Input: part model. Units: mm. Frame: model coordinates. Face numbers are marked on the shaded views. A direction names the side the tool comes from. Coordinates: 2 decimals unless noted, no trailing zeros. Write each loop counter-clockwise with the first axis right and the second up, starting at its lowest first coordinate (ties: lowest second). Pieces come first, ordered by that corner, then holes. Notation, with made-up numbers: (66, 42) - (100, 42) arc R23 cw to (100, 51) - close; hole circle Ø10 at (-5.5, -25.5). An arc over 180 degrees is marked (long way). Put each result on its own line as item: value. Start each with the question number.
1. Cut plane A-A, the plane z = 0. Return loops of the section in (x, y), and give its area (3 significant figures).
2. Pull-direction query (Z, two-part tool) for the marked faces 1, 2, 3 and 4; classes: released by +Z, released by -Z, zero draft, split by the parting line, or undercut.
3. Pin query (flat end, axial travel): pin 1 (2 mm diameter, centred on y = 3.5, z = 9, fed in from -X); pin 2 (5 mm diameter, centred on x = -3.5, z = 2, fed in from -Y); pin 3 (6 mm diameter, centred on x = -3.5, z = 11.5, fed in from -Y); pin 4 (1 mm diameter, centred on x = 3.5, y = 3.5, fed in from +Z). Return the tip coordinate at first contact, or that it passes through.
4. Cut plane C-C, the plane y = -3. Return loops of the section in (x, z).
5. Cut plane D-D, the plane y = 4.5. Return loops of the section in (x, z).
6. Cut plane B-B, the plane x = 0. Return loops of the section in (y, z), and give its area (3 significant figures).
7. Access query for the marked faces 5 and 6. Directions: +Z, -Z, +X, -X, +Y, -Y. A direction counts if a zero-diameter tool reaches every point of the face in a straight line with its end or side. Return the directions, or none.
8. Line query: line 1 (X direction, y = -0.25, z = 0); line 2 (Z direction, x = 1, y = -5.75); line 3 (Y direction, x = 0, z = 11). Output: solid intervals per line, ascending.
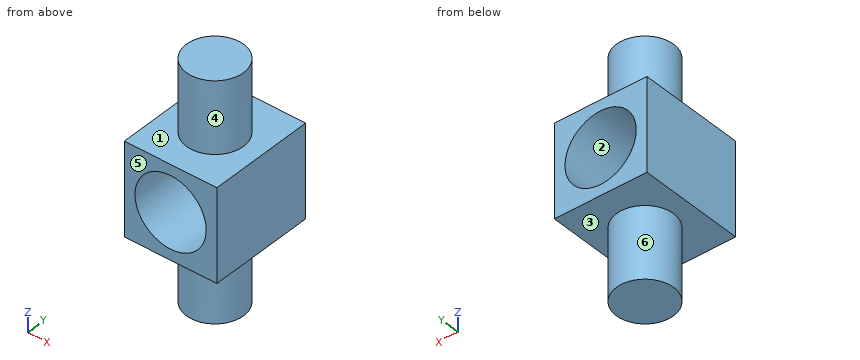
from build123d import *

# Parameters (mm, degrees)
SKETCH1_W           = 13
SKETCH1_H           = 13
SKETCH1_R           = 5
BOSS_EXTRUDE1_DEPTH = 7.5
SKETCH2_R           = 4
BOSS_EXTRUDE2_DEPTH = 10


with BuildPart() as part:
    # Sketch1 → Boss-Extrude1 (new, symmetric)
    with BuildSketch(Plane(origin=(0, 0, 0), x_dir=(1, 0, 0), z_dir=(0, 1, 0))):
        Rectangle(SKETCH1_W, SKETCH1_H)
        with Locations(Location((0, 0, 0), (0, 0, 270))):
            Circle(SKETCH1_R, mode=Mode.SUBTRACT)
    extrude(amount=BOSS_EXTRUDE1_DEPTH, both=True)

    # Sketch2 → Boss-Extrude2 (add)
    with BuildSketch(Plane.XY.offset(6.5)):
        Circle(SKETCH2_R)
    boss_extrude2 = extrude(amount=BOSS_EXTRUDE2_DEPTH)

    # Mirror1: Boss-Extrude2 across plane
    add(boss_extrude2.mirror(Plane.XY))


solid = part.part
Report:
1. outline: (-6.5, -7.5) - (-5, -7.5) - (-5, 7.5) - (-6.5, 7.5) - close; (5, -7.5) - (6.5, -7.5) - (6.5, 7.5) - (5, 7.5) - close
1. area: 45.0 mm^2
2. face 1: released by +Z
2. face 2: undercut
2. face 3: released by -Z
2. face 4: zero draft
3. pin 1: stops at x = -3.12
3. pin 2: stops at y = -7.5
3. pin 3: stops at y = -3.97
3. pin 4: stops at z = 6.5
4. outline: (-6.5, -6.5) - (-2.65, -6.5) - (-2.65, -16.5) - (2.65, -16.5) - (2.65, -6.5) - (6.5, -6.5) - (6.5, 6.5) - (2.65, 6.5) - (2.65, 16.5) - (-2.65, 16.5) - (-2.65, 6.5) - (-6.5, 6.5) - close; hole circle Ø10 at (0, 0)
5. outline: (-6.5, -6.5) - (6.5, -6.5) - (6.5, 6.5) - (-6.5, 6.5) - close; hole circle Ø10 at (0, 0)
6. outline: (-7.5, -6.5) - (-4, -6.5) - (-4, -16.5) - (4, -16.5) - (4, -6.5) - (7.5, -6.5) - (7.5, -5) - (-7.5, -5) - close; (-7.5, 5) - (7.5, 5) - (7.5, 6.5) - (4, 6.5) - (4, 16.5) - (-4, 16.5) - (-4, 6.5) - (-7.5, 6.5) - close
6. area: 205 mm^2
7. face 5: +Z, -Z, +X, -X, -Y
7. face 6: -Z
8. line 1: x = -6.5 to -5, 5 to 6.5
8. line 2: z = -6.5 to -4.9, 4.9 to 6.5
8. line 3: y = -4 to 4
